Drawing for the job (mm, zero at the part's lowest x, y, z). A direction names the side the tool comes from. Round coordinates to 2 decimals unless told otherwise and drop trailing zeros. Loops run counter-clockwise (first coordinate to the right, second up) from the corner with the lowest first, then second, coordinate; pieces in that order, holes last.
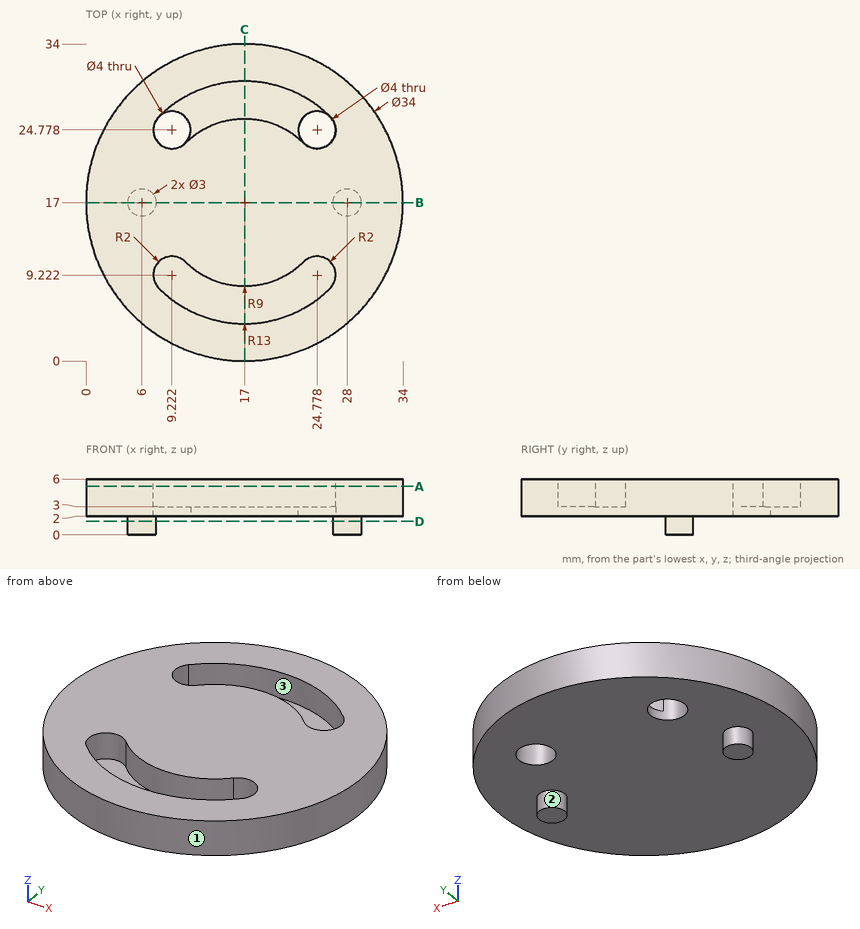
Q1. Tool access for the marked faces 1, 2 and 3: list every direction of +Z, -Z, +X, -X, +Y, -Y with a clear straight run to the whole face (end or side of a thin tool).
Q2. Flat gauge pins, fed straight in: P1, Ø2, axis at x = 19.5, y = 27, coming from the +Z side; P2, Ø6, axis at x = 18, y = 21, coming from the -Z side. Where does each tip first touch, or does it go through?
Q3. Probe line 1 (Y direction, x = 21, z = 4.2); line 2 (Z direction, x = 22, y = 8.5); line 3 (Y direction, x = 12.5, z = 5.45) (1 decimal). List the from-to ranges inside material, lowest first.
Q4. Slice it at A-A on z = 5.2. Give the cut face in (x, y).
Q5. Slice it at D-D on z = 1.45. Give the cut face in (x, y), plus the area to 3 significant figures.
Q6. Slice it at C-C on x = 17. Give the cut face in (y, z), plus the area to 3 significant figures.
Q7. Slice it at B-B on y = 17. Give the cut face in (x, z).
Reply:
1. face 1: +Z, -Z
1. face 2: -Z
1. face 3: +Z
2. P1: stops at z = 3
2. P2: stops at z = 2
3. line 1: y = 0.48 to 4.63, 8.94 to 25.06, 29.37 to 33.52
3. line 2: z = 2 to 3
3. line 3: y = 0.6 to 4.8, 9.2 to 24.8, 29.2 to 33.4
4. outline: circle Ø34 at (17, 17); hole (7.81, 7.81) arc R13 ccw to (26.19, 7.81) arc R2 ccw to (23.36, 10.64) arc R9 cw to (10.64, 10.64) arc R2 ccw to start; hole (7.81, 26.19) arc R2 ccw to (10.64, 23.36) arc R9 cw to (23.36, 23.36) arc R2 ccw to (26.19, 26.19) arc R13 ccw to start
5. outline: circle Ø3 at (6, 17); circle Ø3 at (28, 17)
5. area: 14.1 mm2
6. outline: (0, 2) - (34, 2) - (34, 6) - (30, 6) - (30, 3) - (26, 3) - (26, 6) - (8, 6) - (8, 3) - (4, 3) - (4, 6) - (0, 6) - close
6. area: 112 mm2
7. outline: (0, 2) - (4.5, 2) - (4.5, 0) - (7.5, 0) - (7.5, 2) - (26.5, 2) - (26.5, 0) - (29.5, 0) - (29.5, 2) - (34, 2) - (34, 6) - (0, 6) - close
